Part print with two shaded views. Sizes in mm from the minimum x, y, z corner. A direction names the side the tool comes from. Round coordinates to 2 decimals unless told otherwise and drop trailing zeros. Loops run counter-clockwise (first coordinate to the right, second up) from the corner with the lowest first, then second, coordinate; pieces in that order, holes last. Notation, with made-up numbers: (-13, 5) -> (5, 5) arc R24 cw to (5, 41) -> close; hole circle Ø9 at (66, 71.25). An arc over 180 degrees is marked (long way). Use a Markdown table: item, result. Add a question column.
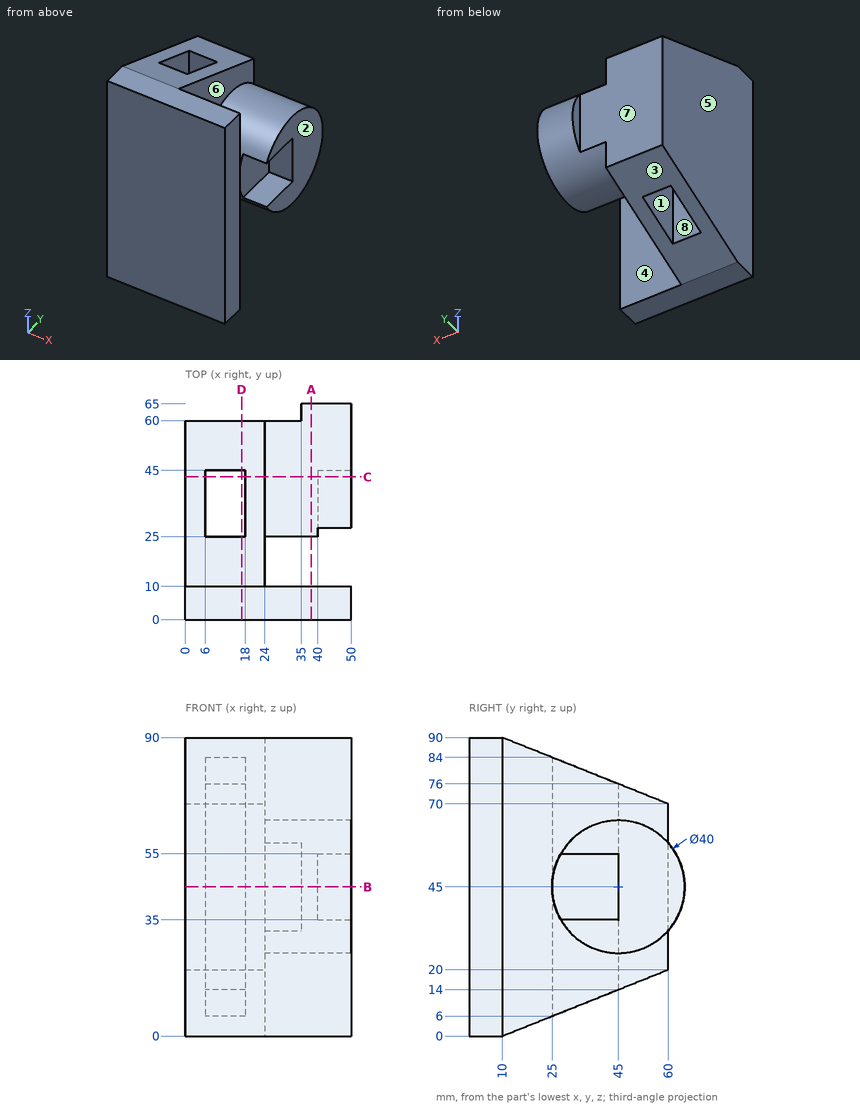
1) Cut at B-B on z = 45. Write the cut outline in (x, y).
2) Cut at C-C on y = 43. Write the cut outline in (x, z), and give its area (3 significant figures).
3) Wall check: probe 1 along X at (y, z) = (37, 36); probe 2 along Y at (x, z) = (37, 30); probe 3 along X at (y, z) = (31.5, 60.5). Give the ranges that are in metal, low to high. Write a range as from..to.
4) Cut at D-D on x = 17. Write the cut outline in (y, z), and give its area (3 significant figures).
5) Cut at A-A on x = 38. Write the cut outline in (y, z).
6) Tool access for the marked faces 4, 5, 6, 7 and 8: list every direction of +Z, -Z, +X, -X, +Y, -Y with a clear straight run to the whole face (end or side of a thin tool).
7) Pin check, flat tips, straight feed: pin 1 Ø8 at (x, z) = (44.5, 47) entering from -Y; pin 2 Ø6 at (x, z) = (11, 43.5) entering from +Y; pin 3 Ø12 at (x, z) = (42, 28.5) entering from +Y; pin 4 Ø1 at (x, z) = (30, 72.5) entering from +Y. Stop position of each tip, or through.
8) Pull direction Y, two halves, no side cores. Call the marked faces 1, 2 and 3: +Y half, -Y half, draft (parallel to the pull), parting line (faces both ways), or undercut.
Established:
| question | item | result |
|---|---|---|
| 1 | outline | (0, 0) -> (50, 0) -> (50, 10) -> (24, 10) -> (24, 25) -> (40, 25) -> (40, 45) -> (50, 45) -> (50, 65) -> (35, 65) -> (35, 60) -> (0, 60) -> close; hole (6, 25) -> (18, 25) -> (18, 45) -> (6, 45) -> close |
| 2 | outline | (0, 13.2) -> (6, 13.2) -> (6, 76.8) -> (0, 76.8) -> close; (18, 13.2) -> (24, 13.2) -> (24, 25.1) -> (50, 25.1) -> (50, 35) -> (40, 35) -> (40, 55) -> (50, 55) -> (50, 64.9) -> (24, 64.9) -> (24, 76.8) -> (18, 76.8) -> close |
| 2 | area | 1,600 mm^2 |
| 3 | probe 1 | x = 0..6, 18..40 |
| 3 | probe 2 | y = 0..10, 31.77..58.23 |
| 3 | probe 3 | x = 0..6, 18..24 |
| 4 | outline | (0, 0) -> (10, 0) -> (25, 6) -> (25, 84) -> (10, 90) -> (0, 90) -> close; (45, 14) -> (60, 20) -> (60, 70) -> (45, 76) -> close |
| 4 | area | 3,000 mm^2 |
| 5 | outline | (0, 0) -> (10, 0) -> (10, 90) -> (0, 90) -> close; circle Ø40 at (45, 45) |
| 6 | face 4 | +Z, -Z, +X |
| 6 | face 5 | +Z, -Z, -X, +Y, -Y |
| 6 | face 6 | +X |
| 6 | face 7 | +Z, -Z, -X, +Y |
| 6 | face 8 | +Z, -Z |
| 7 | pin 1 | stops at y = 0 |
| 7 | pin 2 | stops at y = 60 |
| 7 | pin 3 | stops at y = 62.02 |
| 7 | pin 4 | stops at y = 10 |
| 8 | face 1 | undercut |
| 8 | face 2 | draft |
| 8 | face 3 | +Y half |
